```python
from build123d import *

# Parameters (mm, degrees)
SKETCH_1_R          = 16
EXTRUDE_1_DEPTH     = 20
SKETCH_2_R          = 20
EXTRUDE_2_DEPTH     = 26
SKETCH_3_R          = 16
EXTRUDE_3_DEPTH     = 20
SKETCH_4_R          = 9.5
CUT_EXTRUDE_1_DEPTH = 27
SKETCH_5_R          = 5.5
CUT_EXTRUDE_2_DEPTH = 27
SKETCH_6_R          = 10
CUT_EXTRUDE_3_DEPTH = 12
CUT_EXTRUDE_4_DEPTH = 27
CUT_EXTRUDE_5_DEPTH = 27
CHAMFER_1_SIZE      = 0.3


with BuildPart() as part:
    # 草图1 → 拉伸1 (new body)
    with BuildSketch(Plane(origin=(0, 0, 0), x_dir=(0, -1, 0), z_dir=(0, 0, 1))):
        with Locations(Location((0, 0, 0), (0, 0, 90))):
            Circle(SKETCH_1_R)
    extrude(amount=EXTRUDE_1_DEPTH)

    # 草图2 → 拉伸2 (add)
    with BuildSketch(Plane(origin=(0, 0, 20), x_dir=(0, 1, 0), z_dir=(0, 0, 1))):
        with Locations(Location((0, 0, 0), (0, 0, 90))):
            Circle(SKETCH_2_R)
    extrude(amount=EXTRUDE_2_DEPTH)

    # 草图3 → 拉伸3 (add)
    with BuildSketch(Plane(origin=(0, 0, 46), x_dir=(0, 1, 0), z_dir=(0, 0, 1))):
        with Locations(Location((0, 0, 0), (0, 0, 270))):
            Circle(SKETCH_3_R)
    extrude(amount=EXTRUDE_3_DEPTH)

    # 草图4 → 切除-拉伸1 (cut)
    with BuildSketch(Plane(origin=(0, 0, 0), x_dir=(-1, 0, 0), z_dir=(0, 0, -1))):
        Circle(SKETCH_4_R)
    extrude(amount=-CUT_EXTRUDE_1_DEPTH, mode=Mode.SUBTRACT)

    # 草图5 → 切除-拉伸2 (cut)
    with BuildSketch(Plane.XY.offset(66)):
        Circle(SKETCH_5_R)
    extrude(amount=-CUT_EXTRUDE_2_DEPTH, mode=Mode.SUBTRACT)

    # 草图6 → 切除-拉伸3 (cut)
    with BuildSketch(Plane.XY.offset(39)):
        Circle(SKETCH_6_R)
    extrude(amount=-CUT_EXTRUDE_3_DEPTH, mode=Mode.SUBTRACT)

    # 草图7 → 切除-拉伸4 (cut)
    with BuildSketch(Plane(origin=(0, 0, 0), x_dir=(-1, 0, 0), z_dir=(0, 0, -1))):
        with BuildLine():
            Line((-3, 12), (-3, 9.013878189))
            ThreePointArc((-3, 9.013878189), (0, 9.5), (3, 9.013878189))
            Line((3, 9.013878189), (3, 12))
            Line((3, 12), (-3, 12))
        make_face()
    extrude(amount=-CUT_EXTRUDE_4_DEPTH, mode=Mode.SUBTRACT)

    # 草图8 → 切除-拉伸5 (cut)
    with BuildSketch(Plane.XY.offset(66)):
        with BuildLine():
            Line((-2, 8.5), (-2, 5.123475383))
            ThreePointArc((-2, 5.123475383), (0, 5.5), (2, 5.123475383))
            Line((2, 5.123475383), (2, 8.5))
            Line((2, 8.5), (-2, 8.5))
        make_face()
    extrude(amount=-CUT_EXTRUDE_5_DEPTH, mode=Mode.SUBTRACT)

    # 倒角1
    chamfer_1_edges = [part.edges().sort_by_distance(p)[0] for p in [
        (0, -9.5, 0),
        (0, 12, 0),
        (3, 10.506939094, 0),
        (-3, 10.506939094, 0),
        (0, -5.5, 66),
        (0, 8.5, 66),
        (-2, 6.811737691, 66),
        (2, 6.811737691, 66),
    ]]
    chamfer(chamfer_1_edges, length=CHAMFER_1_SIZE)


solid = part.part
```
Check sheet for the modelled part. Datum: model origin and axes. Units: mm. A direction names the side the tool comes from. Round coordinates to 2 decimals unless told otherwise and drop trailing zeros. Order: outer loops, then holes, each group sorted by start corner. A loop starts at its lowest first (then second) coordinate and runs counter-clockwise, first axis right, second up. Notation, with made-up numbers: (72.25, 16.5) -> (129.25, 16.5) arc R35 cw to (129.25, 53.5) -> close; hole circle Ø6 at (63.25, 12.25). An arc over 180 degrees is marked (long way). Use CSV: the item, a comma, the result in double quotes.
(1) Depth check by flat-ended pin: pin 1 (8 mm diameter, centred on x = 11, z = 13.5, fed in from +Y); pin 2 (2 mm diameter, centred on x = 0.5, y = 10, fed in from -Z); pin 3 (5 mm diameter, centred on y = -9.5, z = 55, fed in from -X). Enter the tip coordinate at first touch or a pass-through.
Worked out:
pin 1,"y = 14.39"
pin 2,"z = 27"
pin 3,"x = -14.39"
(2) Cross-section at D-D (x = -13). Record the boundary of the cut face in (y, z), and give its area (3 significant figures).
Worked out:
outline,"(-15.2, 20) -> (-9.33, 20) -> (-9.33, 0) -> (9.33, 0) -> (9.33, 20) -> (15.2, 20) -> (15.2, 46) -> (9.33, 46) -> (9.33, 66) -> (-9.33, 66) -> (-9.33, 46) -> (-15.2, 46) -> close"
area,"1,540 mm²"
(3) Tool access check on faces 4 (the face through (-2.17, -9.76, 33.08)), 5 (the face through (8.98, -13.43, 46)), 6 (the face through (-2, 7, 53)), 7 (the face through (0, -7, 66)), 8 (the face through (0, 12, 13)). Record the directions out of +Z, -Z, +X, -X, +Y, -Y that give a thin tool (end or side, any length) a straight path to the whole face; none if there is none.
Worked out:
face 4,"none"
face 5,"+Z"
face 6,"+Z, -Z"
face 7,"+Z, +X, -X, +Y, -Y"
face 8,"-Z"
(4) Cross-section at B-B (x = 0). Record the boundary of the cut face in (y, z), and give its area (3 significant figures).
Worked out:
outline,"(-20, 20) -> (-16, 20) -> (-16, 0) -> (-9.8, 0) -> (-9.5, 0.3) -> (-9.5, 27) -> (-10, 27) -> (-10, 39) -> (-5.5, 39) -> (-5.5, 65.7) -> (-5.8, 66) -> (-16, 66) -> (-16, 46) -> (-20, 46) -> close; (8.5, 39) -> (10, 39) -> (10, 27) -> (12, 27) -> (12, 0.3) -> (12.3, 0) -> (16, 0) -> (16, 20) -> (20, 20) -> (20, 46) -> (16, 46) -> (16, 66) -> (8.8, 66) -> (8.5, 65.7) -> close"
area,"1,120 mm²"
(5) Cross-section at A-A (y = 0). Record the boundary of the cut face in (x, z), and give its area (3 significant figures).
Worked out:
outline,"(-20, 20) -> (-16, 20) -> (-16, 0) -> (-9.8, 0) -> (-9.5, 0.3) -> (-9.5, 27) -> (-10, 27) -> (-10, 39) -> (-5.5, 39) -> (-5.5, 65.7) -> (-5.8, 66) -> (-16, 66) -> (-16, 46) -> (-20, 46) -> close; (5.5, 39) -> (10, 39) -> (10, 27) -> (9.5, 27) -> (9.5, 0.3) -> (9.8, 0) -> (16, 0) -> (16, 20) -> (20, 20) -> (20, 46) -> (16, 46) -> (16, 66) -> (5.8, 66) -> (5.5, 65.7) -> close"
area,"1,270 mm²"
(6) Draft check along Y on faces 1 (the face through (-0.38, -9.607, 0.185)), 2 (the face through (-3.47, -15.62, 55.86)), 3 (the face through (8.98, -13.43, 20)). Enter one of: pulls with the +Y half, pulls with the -Y half, needs draft (parallel to the pull), parting line crosses it, or undercut.
Worked out:
face 1,"undercut"
face 2,"parting line crosses it"
face 3,"needs draft"
(7) Cross-section at C-C (z = 14). Record the boundary of the cut face in (x, y), and give its area (3 significant figures).
Worked out:
outline,"circle Ø32 at (0, 0); hole (-3, 9.01) arc R9.5 ccw (long way) to (3, 9.01) -> (3, 12) -> (-3, 12) -> close"
area,"505 mm²"
(8) Material ranges on line 1 along Y through (x, z) = (0, 6.5); line 2 along Y through (x, z) = (0, 34); line 3 along X through (y, z) = (4.5, 60.5), recorded low to high. Write a range as from..to.
Worked out:
line 1,"-16..-9.5, 12..16"
line 2,"-20..-10, 10..20"
line 3,"-15.35..-3.16, 3.16..15.35"
